Input: part model. Units: mm. Frame: model coordinates. Coordinates: 2 decimals unless noted, no trailing zeros. Order: outer loops, then holes, each group sorted by start corner. A loop starts at its lowest first (then second) coordinate and runs counter-clockwise, first axis right, second up. Notation, with made-up numbers: (47.25, 30) -> (54.25, 30) arc R16 ccw to (54.25, 45) -> close; hole circle Ø10 at (-26, 17). An arc over 180 degrees is marked (long way). Use one line per item in the form item = value. Start each with the question number.
1) Section query C-C on z = 0.9. Output: boundary loops of the cut face in (x, y), then the cut area to 3 significant figures.
2) Section query D-D on y = 26. Output: boundary loops of the cut face in (x, z), then the cut area to 3 significant figures.
3) Ray query, line 1 along Y through (x, z) = (-17.5, 0.9); line 2 along Y through (x, z) = (0, 1.25); line 3 along X through (y, z) = (2.5, 0.2). Return the intervals inside material, ascending.
4) Section query A-A on x = -24. Output: boundary loops of the cut face in (y, z).
5) Section query B-B on y = 15. Output: boundary loops of the cut face in (x, z), then the cut area to 3 significant figures.
6) Pin query (flat end, axial travel): pin 1 (3.5 mm diameter, centred on x = 17.5, y = 26, fed in from -Z). Return the tip coordinate at first contact, or that it passes through.
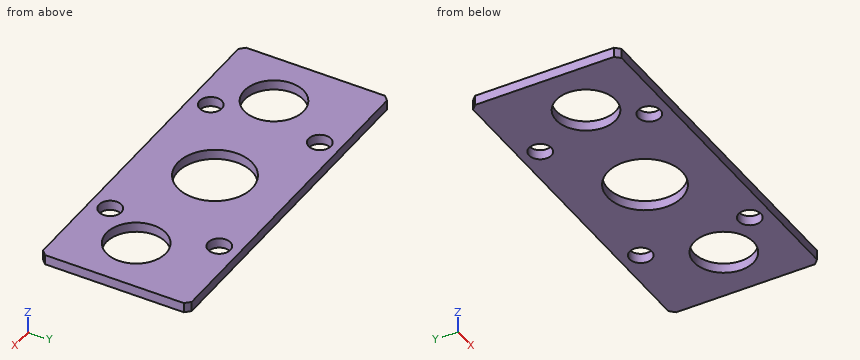
from build123d import *

# Parameters (mm, degrees)
SKETCH1_W                  = 70
SKETCH1_H                  = 30
SKETCH1_R                  = 6
SKETCH1_R_2                = 7.5
BOSS_EXTRUDE1_DEPTH        = 2
F_4_5_4_5_DIAMETER_HOLE1_D = 4.5
CHAMFER1_SIZE              = 1


with BuildPart() as part:
    # Sketch1 → Boss-Extrude1 (new body)
    with BuildSketch(Plane.XY):
        with Locations((0, 15)):
            Rectangle(SKETCH1_W, SKETCH1_H)
        with Locations((-24, 13)):
            Circle(SKETCH1_R, mode=Mode.SUBTRACT)
        with Locations((24, 13)):
            Circle(SKETCH1_R, mode=Mode.SUBTRACT)
        with Locations((0, 15)):
            Circle(SKETCH1_R_2, mode=Mode.SUBTRACT)
    extrude(amount=BOSS_EXTRUDE1_DEPTH)

    # Ø4.5 (4.5) Diameter Hole1 (through all)
    with Locations(Plane.XY.offset(2)):
        with Locations((-17.5, 26), (17.5, 26), (-17.5, 4), (17.5, 4)):
            Hole(F_4_5_4_5_DIAMETER_HOLE1_D / 2)

    # Chamfer1
    chamfer1_edges = [part.edges().sort_by_distance(p)[0] for p in [
        (35, 0, 1),
        (-35, 0, 1),
        (-35, 30, 1),
        (35, 30, 1),
    ]]
    chamfer(chamfer1_edges, length=CHAMFER1_SIZE)


solid = part.part
Answers below:
q1.outline = (-35, 1) -> (-34, 0) -> (34, 0) -> (35, 1) -> (35, 29) -> (34, 30) -> (-34, 30) -> (-35, 29) -> close; hole circle Ø12 at (-24, 13); hole circle Ø4.5 at (-17.5, 4); hole circle Ø4.5 at (-17.5, 26); hole circle Ø15 at (0, 15); hole circle Ø4.5 at (17.5, 4); hole circle Ø4.5 at (17.5, 26); hole circle Ø12 at (24, 13)
q1.area = 1,630 mm^2
q2.outline = (-35, 0) -> (-19.75, 0) -> (-19.75, 2) -> (-35, 2) -> close; (-15.25, 0) -> (15.25, 0) -> (15.25, 2) -> (-15.25, 2) -> close; (19.75, 0) -> (35, 0) -> (35, 2) -> (19.75, 2) -> close
q2.area = 122 mm^2
q3.line_1 = 0 to 1.75, 6.25 to 23.75, 28.25 to 30
q3.line_2 = 0 to 7.5, 22.5 to 30
q3.line_3 = -35 to -19.18, -15.82 to 15.82, 19.18 to 35
q4.outline = (0, 0) -> (7, 0) -> (7, 2) -> (0, 2) -> close; (19, 0) -> (30, 0) -> (30, 2) -> (19, 2) -> close
q5.outline = (-35, 0) -> (-29.66, 0) -> (-29.66, 2) -> (-35, 2) -> close; (-18.34, 0) -> (-7.5, 0) -> (-7.5, 2) -> (-18.34, 2) -> close; (7.5, 0) -> (18.34, 0) -> (18.34, 2) -> (7.5, 2) -> close; (29.66, 0) -> (35, 0) -> (35, 2) -> (29.66, 2) -> close
q5.area = 64.7 mm^2
q6.pin_1 = through
